Read the model definition and answer for the solid it produces. Units are mm, in the model's axes. A direction names the side the tool comes from. Give positions to 0.01 mm unless a question says otherwise; leave off trailing zeros. Loops run counter-clockwise (first coordinate to the right, second up) from the corner with the lowest first, then second, coordinate; pieces in that order, holes last. Notation, with made-up numbers: (-38, -29) -> (-31, -29) arc R19 cw to (-31, -7) -> close; hole circle Ø1 at (36.25, 16.25). An arc over 180 degrees is marked (long way). Answer as CSV lines item,"result". Start each with the question number.
```python
from build123d import *

# Parameters (mm, degrees)
EXTRUDE_390_DEPTH = 12.5
FILLET_1319_R     = 0.8


with BuildPart() as part:
    # 草图1 → Extrude 390 (new body)
    with BuildSketch(Plane(origin=(0, 0, 0), x_dir=(0, 0, -1), z_dir=(1, 0, 0))):
        Polygon((15, 8.660254038), (15, -8.660254038), (0, -17.320508076), (-15, -8.660254038), (-15, 8.660254038), (0, 17.320508076), align=None)
    extrude(amount=EXTRUDE_390_DEPTH)

    # 草图2 → 凸台-旋转1 (revolve)
    with BuildSketch(Plane.XY, mode=Mode.PRIVATE) as revolve_1_sk:
        Polygon((0, 0), (222.5, 0), (222.5, 7.835), (222.5, 10), (170.5, 10), (0, 10), align=None)
    revolve(revolve_1_sk.sketch.rotate(Axis((0, 0, 0), (1, 0, 0)), 90), axis=Axis((0, 0, 0), (1, 0, 0)))

    # 草图3 → 切除-旋转1 (revolve, cut)
    with BuildSketch(Plane.XY):
        Polygon((0, 15), (4.226497308, 22.320508076), (4.226497308, 27.320508076), (-10, 27.320508076), (-10, 15), align=None)
    revolve(axis=Axis((0, 0, 0), (1, 0, 0)), mode=Mode.SUBTRACT)

    # 草图4 → 切除-旋转3 (revolve, cut)
    with BuildSketch(Plane.XY, mode=Mode.PRIVATE) as cut_revolve_3_sk:
        Polygon((12.5, 14.095), (11.7, 14.556880215), (11.7, 17.320508076), (12.5, 17.320508076), align=None)
    revolve(cut_revolve_3_sk.sketch.rotate(Axis((0, 0, 0), (1, 0, 0)), 90), axis=Axis((0, 0, 0), (1, 0, 0)), mode=Mode.SUBTRACT)

    # Fillet 1319
    fillet_1319_edges = [part.edges().sort_by_distance(p)[0] for p in [
        (12.5, 0, -10),
    ]]
    fillet(fillet_1319_edges, radius=FILLET_1319_R)

    # 草图6 → 切除-旋转4 (revolve, cut)
    with BuildSketch(Plane.XY, mode=Mode.PRIVATE) as cut_revolve_4_sk:
        Polygon((221.25, 10), (223.75, 10), (222.5, 7.834936491), align=None)
    revolve(cut_revolve_4_sk.sketch.rotate(Axis((0, 0, 0), (1, 0, 0)), 90), axis=Axis((0, 0, 0), (1, 0, 0)), mode=Mode.SUBTRACT)


solid = part.part
```
(1) Find section A-A on x = 175.5. Write down the section's boundary in (y, z).
(2) A tool of negligible diameter and unlimited length cuts with its end or side. For faces 1 (the face through (5.77, -13.05, 7.4)), 2 (the face through (12.5, -8.3, 7.2)), from which of +Z, -Z, +X, -X, +Y, -Y can it reach the whole face along a straight path? Write none if from no direction.
(3) Find the intervals of material crossed by line 1 along X through (y, z) = (-4.5, -13); line 2 along Y through (x, z) = (143.5, 0.5); line 3 along X through (y, z) = (7.5, 12.5), in increasing order. Write a range as from..to.
(4) Each of these flat-tipped pins is pushed along its axis until it touches: P1, Ø6, axis at x = 187.5, y = -8, coming from the +Z side; P2, Ø1, axis at x = 57, y = -4.5, coming from the -Z side; P3, Ø2, axis at x = 38, z = 3, coming from the -Y side. Where does it stop, or does it pass through?
Answer block:
1,outline,"circle Ø20 at (0, 0)"
2,face 1,"+Z, +X, -X, -Y"
2,face 2,"+X"
3,line 1,"x = 0..12.5"
3,line 2,"y = -9.99..9.99"
3,line 3,"x = 0..11.7"
4,P1,"stops at z = 8.66"
4,P2,"stops at z = -9.17"
4,P3,"stops at y = -9.8"
